Part print with two shaded views. Sizes in mm from the minimum x, y, z corner. A direction names the side the tool comes from. Give positions to 0.01 mm unless a question says otherwise; leave off trailing zeros. Write each loop counter-clockwise with the first axis right and the second up, starting at its lowest first coordinate (ties: lowest second). Pieces come first, ordered by that corner, then holes. Notation, with made-up numbers: (-12.75, -22.75) -> (8.25, -22.75) arc R30 ccw to (8.25, 14.25) -> close; hole circle Ø6 at (17, -20.5). An arc over 180 degrees is marked (long way). Use one line per item in the form item = value. Start each with the question number.
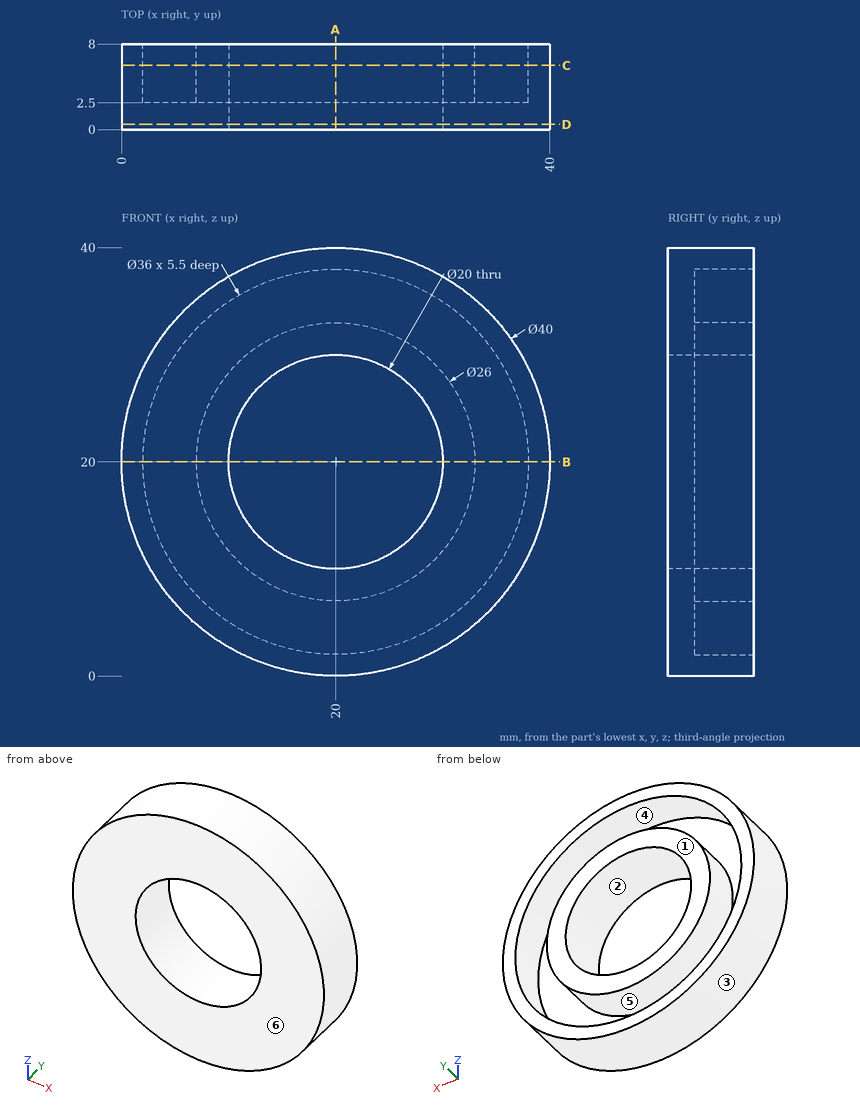
1) Cut at A-A (x = 20). Give the cut face in (y, z), and give its area (3 significant figures).
2) Pin check, flat tips, straight feed: pin 1 (6 mm diameter, centred on x = 20, z = 28.5, fed in from -Y); pin 2 (1.5 mm diameter, centred on x = 21, y = 5, fed in from +Z); pin 3 (1.5 mm diameter, centred on x = 22.5, y = 1.5, fed in from -Z); pin 4 (2 mm diameter, centred on x = 31.5, y = 1.5, fed in from +Z). Stop position of each tip, or through.
3) Cut at C-C (y = 6). Give the cut face in (x, z).
4) Wall check: line 1 along X through (y, z) = (5.4, 20); line 2 along Z through (x, y) = (13, 5) (3 decimals); line 3 along Z through (x, y) = (31.5, 5). Give the ranges that are in metal, low to high. Write a range as from..to.
5) Cut at D-D (y = 0.5). Give the cut face in (x, z).
6) Two-plate mould, pull along X, no slides. Class the marked faces 1, 2, 3 and 4: released by +X, released by -X, zero draft, split by the parting line, or undercut.
7) Cut at B-B (z = 20). Give the cut face in (x, y).
8) 3-axis set-ups, long thin cutter, end or side, ignore diameter. For the marked faces 5 and 6: which of +Z, -Z, +X, -X, +Y, -Y reach the whole face in a straight line?
Final values:
q1.outline = (0, 0) -> (8, 0) -> (8, 2) -> (2.5, 2) -> (2.5, 7) -> (8, 7) -> (8, 10) -> (0, 10) -> close; (0, 30) -> (8, 30) -> (8, 33) -> (2.5, 33) -> (2.5, 38) -> (8, 38) -> (8, 40) -> (0, 40) -> close
q1.area = 105 mm^2
q2.pin_1 = 0
q2.pin_2 = 40
q2.pin_3 = 0.08
q2.pin_4 = 37.02
q3.outline = circle Ø40 at (20, 20); circle Ø26 at (20, 20); hole circle Ø36 at (20, 20); hole circle Ø20 at (20, 20)
q4.line_1 = 0..2, 7..10, 30..33, 38..40
q4.line_2 = 1.265..3.417, 9.046..12.859, 27.141..30.954, 36.583..38.735
q4.line_3 = 3.64..6.15, 13.94..26.06, 33.85..36.36
q5.outline = circle Ø40 at (20, 20); hole circle Ø20 at (20, 20)
q6.face_1 = zero draft
q6.face_2 = undercut
q6.face_3 = split by the parting line
q6.face_4 = undercut
q7.outline = (0, 0) -> (10, 0) -> (10, 8) -> (7, 8) -> (7, 2.5) -> (2, 2.5) -> (2, 8) -> (0, 8) -> close; (30, 0) -> (40, 0) -> (40, 8) -> (38, 8) -> (38, 2.5) -> (33, 2.5) -> (33, 8) -> (30, 8) -> close
q8.face_5 = +Y
q8.face_6 = +Z, -Z, +X, -X, -Y
